```python
from build123d import *

# Parameters (mm, degrees)
SKETCH1_W           = 90
SKETCH1_H           = 70
BOSS_EXTRUDE1_DEPTH = 30
SKETCH2_R           = 17
BOSS_EXTRUDE2_DEPTH = 10
CUT_EXTRUDE1_DEPTH  = 197.38228026


with BuildPart() as part:
    # Sketch1 → Boss-Extrude1 (new body)
    with BuildSketch(Plane(origin=(0, 0, 0), x_dir=(1, 0, 0), z_dir=(0, 1, 0))):
        Rectangle(SKETCH1_W, SKETCH1_H)
    extrude(amount=BOSS_EXTRUDE1_DEPTH)

    # Sketch2 → Boss-Extrude2 (add)
    with BuildSketch(Plane(origin=(45, 0, 0), x_dir=(0, 0, -1), z_dir=(1, 0, 0))):
        with BuildLine():
            Line((-20.861305824, 152.409547532), (-35, 30))
            Line((-35, 30), (35, 30))
            Line((35, 30), (20.861305824, 152.409547532))
            ThreePointArc((20.861305824, 152.409547532), (0, 171), (-20.861305824, 152.409547532))
        make_face()
        with Locations((0, 135)):
            Circle(SKETCH2_R, mode=Mode.SUBTRACT)
    boss_extrude2 = extrude(amount=-BOSS_EXTRUDE2_DEPTH)

    # Mirror1: Boss-Extrude2 across plane
    add(boss_extrude2.mirror(Plane(origin=(0, 0, 0), x_dir=(0, 0, 1), z_dir=(1, 0, 0))))

    # Sketch3 → Cut-Extrude1 (cut, through all)
    with BuildSketch(Plane(origin=(45, 0, 0), x_dir=(0, 0, -1), z_dir=(1, 0, 0))):
        with BuildLine():
            Line((25, 20), (-35, 20))
            Line((-35, 20), (-35, 10))
            Line((-35, 10), (25, 10))
            ThreePointArc((25, 10), (20, 15), (25, 20))
        make_face()
        with BuildLine():
            ThreePointArc((30, 15), (28.535533906, 18.535533906), (25, 20))
            Line((25, 20), (25, 10))
            ThreePointArc((25, 10), (28.535533906, 11.464466094), (30, 15))
        make_face()
        with BuildLine():
            Line((25, 10), (25, 20))
            ThreePointArc((25, 20), (20, 15), (25, 10))
        make_face()
    extrude(amount=-CUT_EXTRUDE1_DEPTH, mode=Mode.SUBTRACT)


solid = part.part
```
Work out the finished part from the listing and answer in its coordinate system (mm). A direction names the side the tool comes from. Give positions to 0.01 mm unless a question says otherwise; leave off trailing zeros. Write each loop counter-clockwise with the first axis right and the second up, starting at its lowest first coordinate (ties: lowest second). Pieces come first, ordered by that corner, then holes. Notation, with made-up numbers: (57, 72.5) - (82, 72.5) arc R35 cw to (82, 108.5) - close; hole circle Ø1 at (-31.5, 38). An arc over 180 degrees is marked (long way). Use one line per item in the form item = value.
1. Determine the mould class of faces 1 (the face through (0, 30, 0)), 2 (the face through (45, 87, 0)), 3 (the face through (-45, 87, 0)) for opening direction X: released by +X, released by -X, zero draft, split by the parting line, or undercut.
Filled in:
face_1 = undercut
face_2 = released by +X
face_3 = released by -X
2. For faces 4 (the face through (1, 10, 5)), 5 (the face through (-35, 86, 0)), 6 (the face through (-1, 0, 0)), determine the directions among +Z, -Z, +X, -X, +Y, -Y from which every point of the face is accessible in a straight line to the end or side of a thin tool.
Filled in:
face_4 = +Z, +X, -X
face_5 = +Z, -Z, +Y
face_6 = +Z, -Z, +X, -X, -Y
3. Consider L1, parallel to Y at x = 39.75, z = 0; L2, parallel to Y at x = -6, z = -14; L3, parallel to X at y = 113, z = 11. Determine where each line is inside the solid, lowest interval first.
Filled in:
L1 = 0 to 10, 20 to 118, 152 to 171
L2 = 0 to 10, 20 to 30
L3 = -45 to -35, 35 to 45
4. A cutting plane is placed at D-D (y = 131.5). Write down the section's boundary in (x, z), and give its area (3 significant figures).
Filled in:
outline = (-45, -23.28) - (-35, -23.28) - (-35, -16.64) - (-45, -16.64) - close; (-45, 16.64) - (-35, 16.64) - (-35, 23.28) - (-45, 23.28) - close; (35, -23.28) - (45, -23.28) - (45, -16.64) - (35, -16.64) - close; (35, 16.64) - (45, 16.64) - (45, 23.28) - (35, 23.28) - close
area = 266 mm^2
5. This flat-tipped pin is pushed along its axis until it touches: pin 1 Ø3 at (x, z) = (26, -9) entering from +Y. Where does it stop, or does it pass through?
Filled in:
pin_1 = 30
6. A cutting plane is placed at C-C (x = -23.5). Write down the section's boundary in (y, z), and give its area (3 significant figures).
Filled in:
outline = (0, -35) - (30, -35) - (30, 35) - (20, 35) - (20, -25) arc R5 cw to (10, -25) - (10, 35) - (0, 35) - close
area = 1,460 mm^2
7. A cutting plane is placed at B-B (y = 74.5). Write down the section's boundary in (x, z), and give its area (3 significant figures).
Filled in:
outline = (-45, -29.86) - (-35, -29.86) - (-35, 29.86) - (-45, 29.86) - close; (35, -29.86) - (45, -29.86) - (45, 29.86) - (35, 29.86) - close
area = 1,190 mm^2
8. A cutting plane is placed at A-A (z = 0). Write down the section's boundary in (x, y), and give its area (3 significant figures).
Filled in:
outline = (-45, 0) - (45, 0) - (45, 10) - (-45, 10) - close; (-45, 20) - (45, 20) - (45, 118) - (35, 118) - (35, 30) - (-35, 30) - (-35, 118) - (-45, 118) - close; (-45, 152) - (-35, 152) - (-35, 171) - (-45, 171) - close; (35, 152) - (45, 152) - (45, 171) - (35, 171) - close
area = 3,940 mm^2
